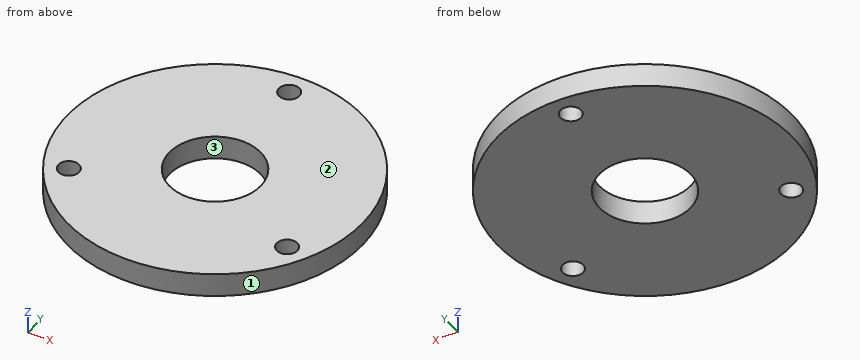
from build123d import *

# Parameters (mm, degrees)
SKETCH1_R           = 50
SKETCH1_R_2         = 3.5
SKETCH1_R_3         = 15.5
BOSS_EXTRUDE1_DEPTH = 8


with BuildPart() as part:
    # Sketch1 → Boss-Extrude1 (new body)
    with BuildSketch(Plane.XY):
        Circle(SKETCH1_R)
        with Locations((0, 42.5)):
            Circle(SKETCH1_R_2, mode=Mode.SUBTRACT)
        with Locations((-36.806079661, -21.25)):
            Circle(SKETCH1_R_2, mode=Mode.SUBTRACT)
        with Locations((36.806079661, -21.25)):
            Circle(SKETCH1_R_2, mode=Mode.SUBTRACT)
        Circle(SKETCH1_R_3, mode=Mode.SUBTRACT)
    extrude(amount=BOSS_EXTRUDE1_DEPTH)


solid = part.part
Can you work these out from the model? Positions are in its coordinate system, mm. Face numbers are marked on the shaded views. Give positions to 0.01 mm unless a question says otherwise; leave off trailing zeros. Order: outer loops, then holes, each group sorted by start corner. A loop starts at its lowest first (then second) coordinate and runs counter-clockwise, first axis right, second up. Notation, with made-up numbers: M 31.5,62 L 83.5,62 A18 cw 83.5,77 Z; hole C -39.5,57.25 d9. An arc over 180 degrees is marked long. One line per item, written item: value.
Item 1: If we section it at D-D on y = -21.25: Write out the boundary of the cut face in (x, z).
Verdict:
outline: M -45.26,0 L -40.31,0 L -40.31,8 L -45.26,8 Z; M -33.31,0 L 33.31,0 L 33.31,8 L -33.31,8 Z; M 40.31,0 L 45.26,0 L 45.26,8 L 40.31,8 Z
Item 2: If we section it at A-A on x = 0: Write out the boundary of the cut face in (y, z).
Verdict:
outline: M -50,0 L -15.5,0 L -15.5,8 L -50,8 Z; M 15.5,0 L 39,0 L 39,8 L 15.5,8 Z; M 46,0 L 50,0 L 50,8 L 46,8 Z
Item 3: If we section it at C-C on x = 36: Write out the boundary of the cut face in (y, z).
Verdict:
outline: M -34.7,0 L -24.66,0 L -24.66,8 L -34.7,8 Z; M -17.84,0 L 34.7,0 L 34.7,8 L -17.84,8 Z
Item 4: For pin 1 (2 mm diameter, centred on x = -13, z = 4.5, fed in from -Y); pin 2 (1 mm diameter, centred on x = 34.5, z = 1.5, fed in from +Y); pin 3 (4 mm diameter, centred on y = -27.5, z = 7, fed in from +X), each with a flat end and sliding along its axis, tell me the tip position at first contact or that it passes through.
Verdict:
pin 1: y = -48.54
pin 2: y = 36.66
pin 3: x = 43.01
Item 5: If we section it at B-B on y = 0: Write out the boundary of the cut face in (x, z), and give its area (3 significant figures).
Verdict:
outline: M -50,0 L -15.5,0 L -15.5,8 L -50,8 Z; M 15.5,0 L 50,0 L 50,8 L 15.5,8 Z
area: 552 mm2
Item 6: If we mould it in two halves opening along Y, with no side actions, what happens to the marked faces 1, 2 and 3? For each: pulls with the +Y half, pulls with the -Y half, needs draft (parallel to the pull), parting line crosses it, or undercut.
Verdict:
face 1: parting line crosses it
face 2: needs draft
face 3: undercut
Item 7: Please list where these lines run through material, in increasing order: line 1 (Y direction, x = 0, z = 2.75); line 2 (X direction, y = -21.5, z = 4); line 3 (X direction, y = -6, z = 4).
Verdict:
line 1: -50 to -15.5, 15.5 to 39, 46 to 50
line 2: -45.14 to -40.3, -33.32 to 33.32, 40.3 to 45.14
line 3: -49.64 to -14.29, 14.29 to 49.64
